The listing builds one solid part. Answer for the finished solid, in the listing's coordinates (mm). Coordinates: 2 decimals unless noted, no trailing zeros. Write each loop counter-clockwise with the first axis right and the second up, starting at its lowest first coordinate (ties: lowest second). Pieces come first, ordered by that corner, then holes.
(1) For a pull along X with two mould halves and no side action, classify faces 1 (the flat face through (-61.93, -36.024, 4.93)), 2 (the flat face through (73.07, 68.976, 4.93)), 3 (the cylindrical face through (38.894, 51.709, 4.93)), 4 (the cylindrical face through (38.894, -21.291, 4.93)) as +X half, -X half, draft (parallel to the pull), parting line (faces both ways), or undercut.
(2) The part is cut by section A-A on x = -7. Determine the outline of the cut face in (y, z).
(3) Straight lines are drawn through the part: line 1 (Y direction, x = 65.5, z = 8); line 2 (Y direction, x = -30, z = 5.5); line 3 (Y direction, x = -34, z = 4). For each, find the intervals that lie inside material, in ascending order.
(4) Given P1, Ø6, axis at x = 67.53, y = 45.51, coming from the +Z side, flat-ended and moving along its own axis, determine where the tip first touches the part or whether it passes through.
(5) The part is cut by section C-C on z = 6.75. Give the number of separate pieces and of enclosed holes in the cut face, plus the area to 3 significant figures.
(6) The part is cut by section D-D on x = -31. Determine the outline of the cut face in (y, z).
(7) The part is cut by section B-B on y = 1. Determine the outline of the cut face in (x, z), plus the area to 3 significant figures.
from build123d import *

# Parameters (mm, degrees)
SKETCH1_W           = 140
SKETCH1_H           = 110
SKETCH1_R           = 3.3
SKETCH1_R_2         = 44
BOSS_EXTRUDE1_DEPTH = 10
M8_TAPPED_HOLE1_D   = 6.8
CHAMFER1_SIZE       = 5
M6_TAPPED_HOLE1_D   = 5


with BuildPart() as part:
    # Sketch1 → Boss-Extrude1 (new body)
    with BuildSketch(Plane.XY):
        with Locations((5.534557186, 16.511254019)):
            Rectangle(SKETCH1_W, SKETCH1_H)
        with Locations((67.534557186, 60.511254019)):
            Circle(SKETCH1_R, mode=Mode.SUBTRACT)
        with Locations((67.534557186, -27.488745981)):
            Circle(SKETCH1_R, mode=Mode.SUBTRACT)
        with Locations((-56.465442814, -27.488745981)):
            Circle(SKETCH1_R, mode=Mode.SUBTRACT)
        with Locations((-56.465442814, 60.511254019)):
            Circle(SKETCH1_R, mode=Mode.SUBTRACT)
        with Locations((5.534557186, 16.511254019)):
            Circle(SKETCH1_R_2, mode=Mode.SUBTRACT)
    extrude(amount=BOSS_EXTRUDE1_DEPTH)

    # M8 Tapped Hole1 (through all)
    with Locations(Plane.XY.offset(10)):
        with Locations((-30.965442814, 53.011254019), (42.034557186, 53.011254019), (42.034557186, -19.988745981), (-30.965442814, -19.988745981)):
            Hole(M8_TAPPED_HOLE1_D / 2)

    # Chamfer1
    chamfer1_edges = [part.edges().sort_by_distance(p)[0] for p in [
        (75.534557186, -38.488745981, 5),
        (-64.465442814, -38.488745981, 5),
        (-64.465442814, 71.511254019, 5),
        (75.534557186, 71.511254019, 5),
    ]]
    chamfer(chamfer1_edges, length=CHAMFER1_SIZE)

    # M6 Tapped Hole1 (through all)
    with Locations(Plane.XY.offset(10)):
        with Locations((67.534557186, 45.511254019), (67.534557186, 29.511254019)):
            Hole(M6_TAPPED_HOLE1_D / 2)


solid = part.part
Model answer:
1. face 1: -X half
1. face 2: +X half
1. face 3: undercut
1. face 4: undercut
2. outline: (-38.49, 0) - (-25.67, 0) - (-25.67, 10) - (-38.49, 10) - close; (58.69, 0) - (71.51, 0) - (71.51, 10) - (58.69, 10) - close
3. line 1: y = -38.49 to -30.09, -24.89 to 28.06, 30.96 to 44.06, 46.96 to 57.91, 63.11 to 71.51
3. line 2: y = -38.49 to -23.25, -16.73 to -9.44, 42.46 to 49.75, 56.27 to 71.51
3. line 3: y = -38.49 to -21.52, -18.46 to -2.8, 35.82 to 51.48, 54.54 to 71.51
4. P1: stops at z = 10
5. separate pieces: 1
5. enclosed holes: 11
5. area: 8,950 mm2
6. outline: (-38.49, 0) - (-23.39, 0) - (-23.39, 10) - (-38.49, 10) - close; (-16.59, 0) - (-8.01, 0) - (-8.01, 10) - (-16.59, 10) - close; (41.03, 0) - (49.61, 0) - (49.61, 10) - (41.03, 10) - close; (56.41, 0) - (71.51, 0) - (71.51, 10) - (56.41, 10) - close
7. outline: (-64.47, 0) - (-35.64, 0) - (-35.64, 10) - (-64.47, 10) - close; (46.71, 0) - (75.53, 0) - (75.53, 10) - (46.71, 10) - close
7. area: 576 mm2
